from build123d import *

# Parameters (mm, degrees)
SKETCH1_W           = 115
SKETCH1_H           = 20
BOSS_EXTRUDE1_DEPTH = 3
SKETCH2_W           = 3
SKETCH2_H           = 20
BOSS_EXTRUDE2_DEPTH = 15
FILLET1_R           = 2
FILLET2_R           = 5
M3_TAPPED_HOLE1_D   = 2.5
FILLET3_R           = 5


with BuildPart() as part:
    # Sketch1 → Boss-Extrude1 (new body)
    with BuildSketch(Plane(origin=(0, 0, 0), x_dir=(1, 0, 0), z_dir=(0, 1, 0))):
        Rectangle(SKETCH1_W, SKETCH1_H)
    extrude(amount=BOSS_EXTRUDE1_DEPTH)

    # Sketch2 → Boss-Extrude2 (add)
    with BuildSketch(Plane(origin=(0, 3, 0), x_dir=(1, 0, 0), z_dir=(0, 1, 0))):
        with Locations((-56, 0)):
            Rectangle(SKETCH2_W, SKETCH2_H)
        with Locations((56, 0)):
            Rectangle(SKETCH2_W, SKETCH2_H)
    extrude(amount=BOSS_EXTRUDE2_DEPTH)

    # Fillet1
    fillet1_edges = [part.edges().sort_by_distance(p)[0] for p in [
        (-54.5, 3, 0),
        (54.5, 3, 0),
    ]]
    fillet(fillet1_edges, radius=FILLET1_R)

    # Fillet2
    fillet2_edges = [part.edges().sort_by_distance(p)[0] for p in [
        (-57.5, 0, 0),
        (57.5, 0, 0),
    ]]
    fillet(fillet2_edges, radius=FILLET2_R)

    # M3 Tapped Hole1 (through all)
    with Locations(Plane.ZY.offset(57.5)):
        with Locations((0, 14), (0, 9)):
            Hole(M3_TAPPED_HOLE1_D / 2)

    # Fillet3
    fillet3_edges = [part.edges().sort_by_distance(p)[0] for p in [
        (-56, 18, 10),
        (-56, 18, -10),
        (56, 18, -10),
        (56, 18, 10),
    ]]
    fillet(fillet3_edges, radius=FILLET3_R)


solid = part.part
Can you work these out from the model? Positions are in its coordinate system, mm. A direction names the side the tool comes from. Coordinates: 2 decimals unless noted, no trailing zeros. Write each loop counter-clockwise with the first axis right and the second up, starting at its lowest first coordinate (ties: lowest second). Pieces come first, ordered by that corner, then holes. Notation, with made-up numbers: (-15.75, -5.75) -> (-3.75, -5.75) arc R26 ccw to (-3.75, 30.25) -> close; hole circle Ø7 at (-30, 48). An arc over 180 degrees is marked (long way). Write item = value, one per line.
(1) Imagine slicing it at A-A (z = 0). Please give me the cut outline in (x, y), and give its area (3 significant figures).
Verdict:
outline = (-57.5, 5) arc R5 ccw to (-52.5, 0) -> (52.5, 0) arc R5 ccw to (57.5, 5) -> (57.5, 7.75) -> (54.5, 7.75) -> (54.5, 5) arc R2 cw to (52.5, 3) -> (-52.5, 3) arc R2 cw to (-54.5, 5) -> (-54.5, 7.75) -> (-57.5, 7.75) -> close; (-57.5, 10.25) -> (-54.5, 10.25) -> (-54.5, 12.75) -> (-57.5, 12.75) -> close; (-57.5, 15.25) -> (-54.5, 15.25) -> (-54.5, 18) -> (-57.5, 18) -> close; (54.5, 10.25) -> (57.5, 10.25) -> (57.5, 12.75) -> (54.5, 12.75) -> close; (54.5, 15.25) -> (57.5, 15.25) -> (57.5, 18) -> (54.5, 18) -> close
area = 396 mm^2
(2) On a 3-axis mill with a long thin cutter (end or side, diameter ignored), from which of +Z, -Z, +X, -X, +Y, -Y can I reach the whole of each face in a straight line? I mean faces 1 (the face through (-53.9, 3.57, -0.14)), 2 (the face through (-56, 16, 9)). Say none if no direction works.
Verdict:
face_1 = +Z, -Z, +Y
face_2 = +Z, +X, -X, +Y
(3) Imagine slicing it at D-D (z = -6.25). Please give me the cut outline in (x, y).
Verdict:
outline = (-57.5, 5) arc R5 ccw to (-52.5, 0) -> (52.5, 0) arc R5 ccw to (57.5, 5) -> (57.5, 17.84) -> (54.5, 17.84) -> (54.5, 5) arc R2 cw to (52.5, 3) -> (-52.5, 3) arc R2 cw to (-54.5, 5) -> (-54.5, 17.84) -> (-57.5, 17.84) -> close
(4) For pin 1 (3 mm diameter, centred on y = 9, z = 0, fed in from -X); pin 2 (10 mm diameter, centred on x = -5.5, z = 3, fed in from +Y), each with a flat end and sliding along its axis, tell me the tip position at first contact or that it passes through.
Verdict:
pin_1 = -57.5
pin_2 = 3
(5) Imagine slicing it at C-C (y = 14). Please give me the cut outline in (x, z).
Verdict:
outline = (-57.5, -9.9) -> (-54.5, -9.9) -> (-54.5, -1.25) -> (-57.5, -1.25) -> close; (-57.5, 1.25) -> (-54.5, 1.25) -> (-54.5, 9.9) -> (-57.5, 9.9) -> close; (54.5, -9.9) -> (57.5, -9.9) -> (57.5, -1.25) -> (54.5, -1.25) -> close; (54.5, 1.25) -> (57.5, 1.25) -> (57.5, 9.9) -> (54.5, 9.9) -> close
(6) Thinking about a two-plate mould opening in X: for faces 3 (the face through (56.02, 10.24, 0.16)), 4 (the face through (-57.5, 11, 0)), 5 (the face through (53.93, 3.6, -0.14)), which applies, +X half, -X half, draft (parallel to the pull), parting line (faces both ways), or undercut?
Verdict:
face_3 = draft
face_4 = -X half
face_5 = undercut
(7) If I drill on probe 1 along X at (y, z) = (9.5, -8.5); probe 2 along Y at (x, z) = (-56.75, 0); probe 3 along Y at (x, z) = (55.85, 0), over which ranges is the centre line in solid material (lowest first)?
Verdict:
probe_1 = -57.5 to -54.5, 54.5 to 57.5
probe_2 = 2.37 to 7.75, 10.25 to 12.75, 15.25 to 18
probe_3 = 1.29 to 7.75, 10.25 to 12.75, 15.25 to 18
(8) Imagine slicing it at B-B (y = 9). Please give me the cut outline in (x, z).
Verdict:
outline = (-57.5, -10) -> (-54.5, -10) -> (-54.5, -1.25) -> (-57.5, -1.25) -> close; (-57.5, 1.25) -> (-54.5, 1.25) -> (-54.5, 10) -> (-57.5, 10) -> close; (54.5, -10) -> (57.5, -10) -> (57.5, -1.25) -> (54.5, -1.25) -> close; (54.5, 1.25) -> (57.5, 1.25) -> (57.5, 10) -> (54.5, 10) -> close
